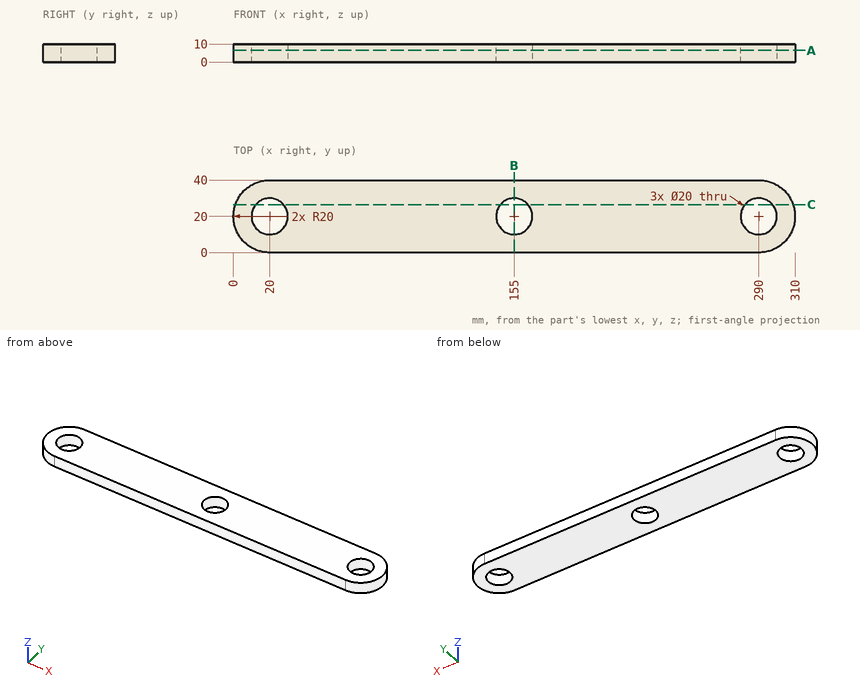
Can you work these out from the drawing? Everything is in mm from the part's minimum corner. Coordinates: 2 decimals unless noted, no trailing zeros. Loops run counter-clockwise (first coordinate to the right, second up) from the corner with the lowest first, then second, coordinate; pieces in that order, holes last.
1) Imagine slicing it at B-B on x = 155. List the corners of the cut face in (y, z) for me, plus the area to 3 significant figures.
2) I need wall thicknesses on probe 1 along X at (y, z) = (21, 5); probe 2 along X at (y, z) = (26, 1.25); probe 3 along Y at (x, z) = (155, 5.75). Which ranges of each line are inside material? Lowest first, please.
3) Imagine slicing it at C-C on y = 26.5. List the corners of the cut face in (x, z) for me, plus the area to 3 significant figures.
4) For pin 1 (3 mm diameter, centred on x = 69.5, z = 5, fed in from -Y); pin 2 (1.5 mm diameter, centred on y = 34, z = 2, fed in from +X), each with a flat end and sliding along its axis, tell me the tip position at first contact or that it passes through.
5) Imagine slicing it at A-A on z = 6.5. List the corners of the cut face in (x, y) for me.
Completed:
1. outline: (0, 0) - (10, 0) - (10, 10) - (0, 10) - close; (30, 0) - (40, 0) - (40, 10) - (30, 10) - close
1. area: 200 mm2
2. probe 1: x = 0.03 to 10.05, 29.95 to 145.05, 164.95 to 280.05, 299.95 to 309.97
2. probe 2: x = 0.92 to 12, 28 to 147, 163 to 282, 298 to 309.08
2. probe 3: y = 0 to 10, 30 to 40
3. outline: (1.09, 0) - (12.4, 0) - (12.4, 10) - (1.09, 10) - close; (27.6, 0) - (147.4, 0) - (147.4, 10) - (27.6, 10) - close; (162.6, 0) - (282.4, 0) - (282.4, 10) - (162.6, 10) - close; (297.6, 0) - (308.91, 0) - (308.91, 10) - (297.6, 10) - close
3. area: 2,620 mm2
4. pin 1: stops at y = 0
4. pin 2: stops at x = 304.98
5. outline: (20, 0) - (290, 0) arc R20 ccw to (290, 40) - (20, 40) arc R20 ccw to start; hole circle Ø20 at (20, 20); hole circle Ø20 at (155, 20); hole circle Ø20 at (290, 20)
